Build history of the part. All positions in model axes, mm. Round coordinates to 2 decimals unless told otherwise and drop trailing zeros. Write each loop counter-clockwise with the first axis right and the second up, starting at its lowest first coordinate (ties: lowest second). Pieces come first, ordered by that corner, then holes.
1) Flat gauge pins, fed straight in: pin 1 (5.5 mm diameter, centred on x = 733.5, y = 16, fed in from +Z); pin 2 (2.5 mm diameter, centred on x = 60.5, y = 16, fed in from +Z); pin 3 (2.5 mm diameter, centred on x = 747, y = 15.5, fed in from -Z); pin 4 (5 mm diameter, centred on y = 5.5, z = -17.5, fed in from +X). Where does each tip first touch, or does it go through?
2) Saw through at A-A (y = 7). Write the cut outline in (x, z) (3 decimals), plus the area to 3 significant figures.
3) Wall check: probe 1 along X at (y, z) = (17, 10); probe 2 along X at (y, z) = (-17, 11.5); probe 3 along Y at (x, z) = (461.5, -2.5). Give the ranges that are in metal, low to high.
4) Saw through at B-B (x = 386). Write the cut outline in (y, z), plus the area to 3 significant figures.
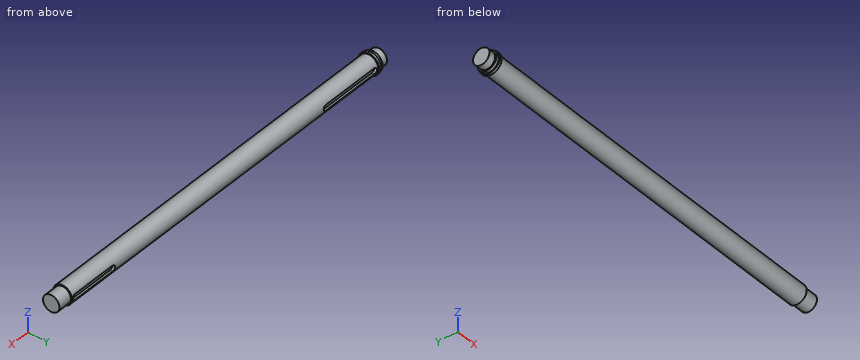
from build123d import *

# Parameters (mm, degrees)
SKETCH_1_R          = 20
EXTRUDE_1_DEPTH     = 803
SKETCH_2_R          = 17.5
EXTRUDE_2_DEPTH     = 30
SKETCH_3_R          = 22.5
EXTRUDE_3_DEPTH     = 5
SKETCH_4_R          = 20.5
EXTRUDE_4_DEPTH     = 6
EXTRUDE_START       = 15
SKETCH_5_R          = 17.5
EXTRUDE_5_DEPTH     = 15
CUT_EXTRUDE_1_DEPTH = 5.92


with BuildPart() as part:
    # 草图1 → 凸台-拉伸1 (new body)
    with BuildSketch(Plane(origin=(0, 0, 0), x_dir=(0, 0, -1), z_dir=(1, 0, 0))):
        Circle(SKETCH_1_R)
    extrude(amount=EXTRUDE_1_DEPTH)

    # 草图2 → 凸台-拉伸2 (add)
    with BuildSketch(Plane(origin=(803, 0, 0), x_dir=(0, 0, -1), z_dir=(1, 0, 0))):
        Circle(SKETCH_2_R)
    extrude(amount=EXTRUDE_2_DEPTH)

    # 草图3 → 凸台-拉伸3 (add)
    with BuildSketch(Plane.ZY):
        Circle(SKETCH_3_R)
    extrude(amount=EXTRUDE_3_DEPTH)

    # 草图4 → 凸台-拉伸4 (add)
    with BuildSketch(Plane.ZY.offset(5)):
        Circle(SKETCH_4_R)
    extrude(amount=EXTRUDE_4_DEPTH)

    # 草图5 → 凸台-拉伸5 (add)
    with BuildSketch(Plane.ZY.offset(11).offset(EXTRUDE_START)):
        with Locations(Location((0, 0, 0), (0, 0, 180))):
            Circle(SKETCH_5_R)
    extrude(amount=-EXTRUDE_5_DEPTH)

    # 草图6 → 切除-拉伸1 (cut)
    with BuildSketch(Plane(origin=(0, 20, 0), x_dir=(1, 0, 0), z_dir=(0, 1, 0))):
        with BuildLine():
            Line((9, 6), (137, 6))
            ThreePointArc((137, 6), (143, 0), (137, -6))
            Line((137, -6), (9, -6))
            ThreePointArc((9, -6), (3, 0), (9, 6))
        make_face()
        with BuildLine():
            Line((794, -6), (696, -6))
            ThreePointArc((696, -6), (690, 0), (696, 6))
            Line((696, 6), (794, 6))
            ThreePointArc((794, 6), (800, 0), (794, -6))
        make_face()
    extrude(amount=-CUT_EXTRUDE_1_DEPTH, mode=Mode.SUBTRACT)


solid = part.part
Evaluation:
1. pin 1: stops at z = 14.98
1. pin 2: stops at z = 13.51
1. pin 3: stops at z = -14.03
1. pin 4: stops at x = 833
2. outline: (-26, -16.039) - (-11, -16.039) - (-11, -19.268) - (-5, -19.268) - (-5, -21.383) - (0, -21.383) - (0, -18.735) - (803, -18.735) - (803, -16.039) - (833, -16.039) - (833, 16.039) - (803, 16.039) - (803, 18.735) - (0, 18.735) - (0, 21.383) - (-5, 21.383) - (-5, 19.268) - (-11, 19.268) - (-11, 16.039) - (-26, 16.039) - close
2. area: 32,000 mm2
3. probe 1: x = -11 to 803
3. probe 2: x = -5 to 0
3. probe 3: y = -19.84 to 19.84
4. outline: circle Ø40 at (0, 0)
4. area: 1,260 mm2
